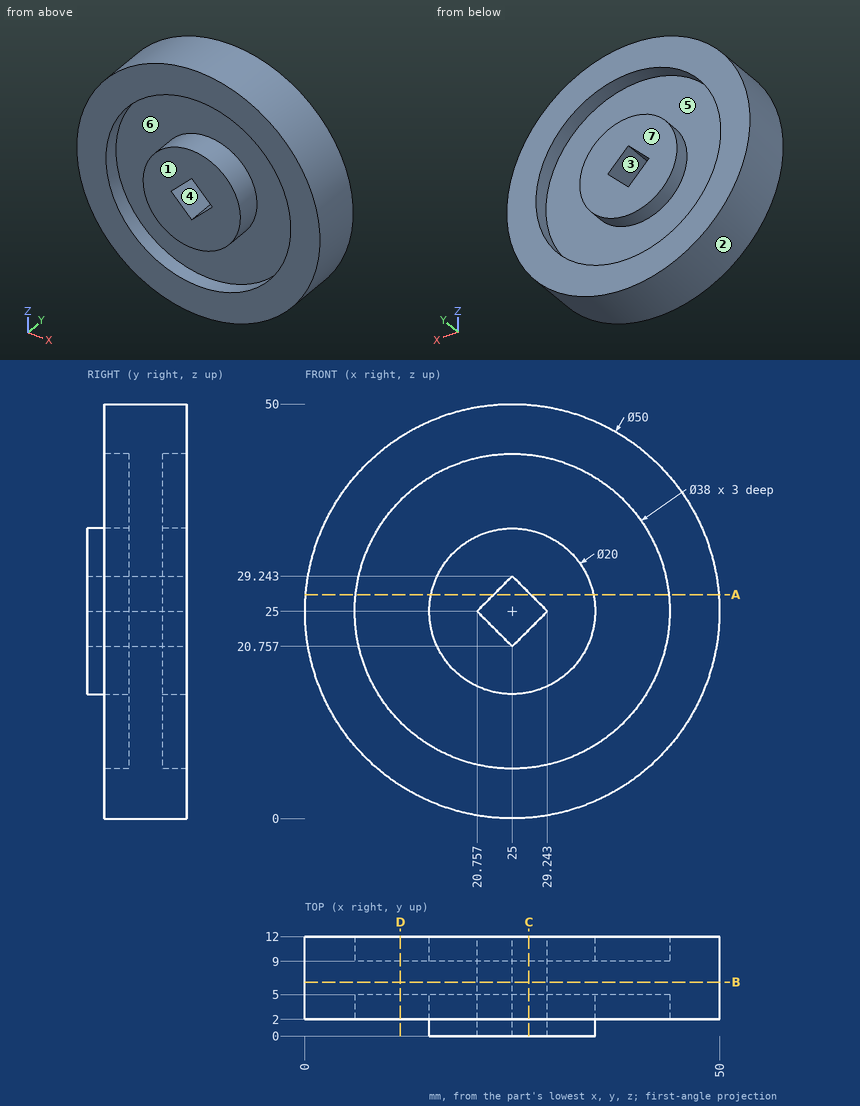
Study the drawing (mm; zero at the part's minimum x, y, z) and answer. A direction names the side the tool comes from. Give positions to 0.01 mm unless a question says otherwise; leave off trailing zeros. Order: outer loops, then holes, each group sorted by start corner. A loop starts at its lowest first (then second) coordinate and runs counter-clockwise, first axis right, second up. Notation, with made-up numbers: (-9.5, 29.25) - (32.5, 29.25) arc R16 ccw to (32.5, 33.25) - close; hole circle Ø3 at (-6, -23.5). An arc over 180 degrees is marked (long way). Answer as CSV lines item,"result". Start each with the question number.
Q1. For the marked faces 5, 6 and 7, determine the directions among +Z, -Z, +X, -X, +Y, -Y from which every point of the face is accessible in a straight line to the end or side of a thin tool.
Q2. Given pin 1 Ø3 at (x, y) = (8.5, 4.5) entering from -Z; pin 2 Ø3 at (x, y) = (20, 4) entering from +Z; pin 3 Ø4 at (y, z) = (1.5, 43) entering from +X (1 decimal), each flat-ended and moving along its own axis, determine where each tip first touches the part or whether it passes through.
Q3. The part is cut by section B-B (y = 6.5). Write down the section's boundary in (x, z).
Q4. The mould has two halves that part along X. Classify the marked faces 1, 2, 3 and 4: +X half, -X half, draft (parallel to the pull), parting line (faces both ways), or undercut.
Q5. Find the intervals of material crossed by L1, parallel to Z at x = 21, y = 10 (1 decimal); L2, parallel to Y at x = 23.5, z = 46; L3, parallel to Y at x = 11, z = 24, in increasing order. Write a range as [from, to].
Q6. The part is cut by section A-A (z = 27). Write down the section's boundary in (x, y) (1 decimal).
Q7. The part is cut by section C-C (x = 27). Write down the section's boundary in (y, z) (1 decimal).
Q8. The part is cut by section D-D (x = 11.5). Write down the section's boundary in (y, z), then the cut area to 3 significant figures.
Check result:
1,face 5,"+Y"
1,face 6,"-Y"
1,face 7,"+Z, -Z, +X, -X, +Y"
2,pin 1,"stops at z = 5"
2,pin 2,"stops at z = 49.75"
2,pin 3,"stops at x = 44.2"
3,outline,"circle Ø50 at (25, 25); hole (20.76, 25) - (25, 20.76) - (29.24, 25) - (25, 29.24) - close"
4,face 1,"draft"
4,face 2,"parting line"
4,face 3,"undercut"
4,face 4,"undercut"
5,L1,"z = [0.3, 6.4], [15.8, 24.8], [25.2, 34.2], [43.6, 49.7]"
5,L2,"y = [2, 12]"
5,L3,"y = [5, 9]"
6,outline,"(0.1, 2) - (6.1, 2) - (6.1, 5) - (15.2, 5) - (15.2, 0) - (22.8, 0) - (22.8, 12) - (15.2, 12) - (15.2, 9) - (6.1, 9) - (6.1, 12) - (0.1, 12) - close; (27.2, 0) - (34.8, 0) - (34.8, 5) - (43.9, 5) - (43.9, 2) - (49.9, 2) - (49.9, 12) - (43.9, 12) - (43.9, 9) - (34.8, 9) - (34.8, 12) - (27.2, 12) - close"
7,outline,"(0, 15.2) - (5, 15.2) - (5, 6.1) - (2, 6.1) - (2, 0.1) - (12, 0.1) - (12, 6.1) - (9, 6.1) - (9, 15.2) - (12, 15.2) - (12, 22.8) - (0, 22.8) - close; (0, 27.2) - (12, 27.2) - (12, 34.8) - (9, 34.8) - (9, 43.9) - (12, 43.9) - (12, 49.9) - (2, 49.9) - (2, 43.9) - (5, 43.9) - (5, 34.8) - (0, 34.8) - close"
8,outline,"(2, 3.96) - (12, 3.96) - (12, 11.63) - (9, 11.63) - (9, 38.37) - (12, 38.37) - (12, 46.04) - (2, 46.04) - (2, 38.37) - (5, 38.37) - (5, 11.63) - (2, 11.63) - close"
8,area,"260 mm²"
